Can you work these out from the model? Positions are in its coordinate system, mm. A direction names the side the tool comes from. Coordinates: 2 decimals unless noted, no trailing zeros. Loops run counter-clockwise (first coordinate to the right, second up) from the corner with the lowest first, then second, coordinate; pieces in that order, holes last.
```python
from build123d import *

# Parameters (mm, degrees)
SKETCH1_R                                           = 90
SKETCH1_R_2                                         = 35
BOSS_EXTRUDE1_DEPTH                                 = 20
CUT_EXTRUDE1_DEPTH                                  = 10
CHAMFER1_SIZE                                       = 5
CSK_FOR_1_4_FLAT_HEAD_MACHINE_SCREW_100_D           = 7.14248
CSK_FOR_1_4_FLAT_HEAD_MACHINE_SCREW_100_CSINK_D     = 12.8778
CSK_FOR_1_4_FLAT_HEAD_MACHINE_SCREW_100_CSINK_ANGLE = 100
MIRROR2_COPY_1_D                                    = 7.14248
MIRROR2_COPY_1_CSINK_D                              = 12.8778
MIRROR2_COPY_1_CSINK_ANGLE                          = 100


with BuildPart() as part:
    # Sketch1 → Boss-Extrude1 (new body)
    with BuildSketch(Plane.XY):
        Circle(SKETCH1_R)
        Circle(SKETCH1_R_2, mode=Mode.SUBTRACT)
    extrude(amount=BOSS_EXTRUDE1_DEPTH)

    # Sketch2 → Cut-Extrude1 (cut)
    with BuildSketch(Plane.XY.offset(20)):
        with BuildLine():
            Line((-19.468288874, 43.327078465), (-30.54243357, 66.327225141))
            ThreePointArc((-30.54243357, 66.327225141), (-53.118804443, 50.105225854), (-67.996083401, 26.620925706))
            Line((-67.996083401, 26.620925706), (-43.882710923, 18.181245339))
            ThreePointArc((-43.882710923, 18.181245339), (-34.079547015, 33.088283051), (-19.468288874, 43.327078465))
        make_face()
        with BuildLine():
            Line((43.882710923, 18.181245339), (67.996083401, 26.620925706))
            ThreePointArc((67.996083401, 26.620925706), (53.118804443, 50.105225854), (30.54243357, 66.327225141))
            Line((30.54243357, 66.327225141), (19.468288874, 43.327078465))
            ThreePointArc((19.468288874, 43.327078465), (34.079547015, 33.088283051), (43.882710923, 18.181245339))
        make_face()
        with BuildLine():
            Line((19.468288874, -43.327078465), (30.54243357, -66.327225141))
            ThreePointArc((30.54243357, -66.327225141), (53.118804443, -50.105225854), (67.996083401, -26.620925706))
            Line((67.996083401, -26.620925706), (43.882710923, -18.181245339))
            ThreePointArc((43.882710923, -18.181245339), (34.079547015, -33.088283051), (19.468288874, -43.327078465))
        make_face()
        with BuildLine():
            Line((-43.882710923, -18.181245339), (-67.996083401, -26.620925706))
            ThreePointArc((-67.996083401, -26.620925706), (-53.118804443, -50.105225854), (-30.54243357, -66.327225141))
            Line((-30.54243357, -66.327225141), (-19.468288874, -43.327078465))
            ThreePointArc((-19.468288874, -43.327078465), (-34.079547015, -33.088283051), (-43.882710923, -18.181245339))
        make_face()
    extrude(amount=-CUT_EXTRUDE1_DEPTH, mode=Mode.SUBTRACT)

    # Chamfer1
    chamfer1_edges = [part.edges().sort_by_distance(p)[0] for p in [
        (-90, 0, 20),
    ]]
    chamfer(chamfer1_edges, length=CHAMFER1_SIZE)

    # CSK for 1/4 Flat Head Machine Screw (100)1 (through all)
    with Locations(Plane.XY.offset(10)):
        with Locations((-42.426406871, 42.426406871)):
            csk_for_1_4_flat_head_machine_screw_100 = CounterSinkHole(CSK_FOR_1_4_FLAT_HEAD_MACHINE_SCREW_100_D / 2, CSK_FOR_1_4_FLAT_HEAD_MACHINE_SCREW_100_CSINK_D / 2, counter_sink_angle=CSK_FOR_1_4_FLAT_HEAD_MACHINE_SCREW_100_CSINK_ANGLE)

    # Mirror1: CSK for 1/4 Flat Head Machine Screw (100)1 across plane
    add(csk_for_1_4_flat_head_machine_screw_100.mirror(Plane(origin=(0, 0, 0), x_dir=(0, 0, 1), z_dir=(1, 0, 0))), mode=Mode.SUBTRACT)

    # Mirror2: CSK for 1/4 Flat Head Machine Screw (100)1 across plane
    add(csk_for_1_4_flat_head_machine_screw_100.mirror(Plane.ZX), mode=Mode.SUBTRACT)

    # Mirror2 copy 1 (through all)
    with Locations(Plane(origin=(0, 0, 10), x_dir=(-1, 0, 0), z_dir=(0, 0, 1))):
        with Locations((-42.426406871, 42.426406871)):
            CounterSinkHole(MIRROR2_COPY_1_D / 2, MIRROR2_COPY_1_CSINK_D / 2, counter_sink_angle=MIRROR2_COPY_1_CSINK_ANGLE)


solid = part.part
```
Item 1: Suppose I cut it at A-A, the plane x = 0. Please give me the cut outline in (y, z), plus the area to 4 significant figures.
Results are:
outline: (-90, 0) - (-35, 0) - (-35, 20) - (-85, 20) - (-90, 15) - close; (35, 0) - (90, 0) - (90, 15) - (85, 20) - (35, 20) - close
area: 2,175 mm2
Item 2: I'm going to push flat-ended pins straight in: P1, Ø10, axis at x = -61.5, z = 12, coming from the -Y side; P2, Ø12, axis at y = 40.5, z = 15.5, coming from the -X side; P3, Ø10, axis at x = -1.5, y = 25, coming from the -Z side; P4, Ø3, axis at x = 12, z = 14, coming from the +Y side. Where does each tip first touch, or does it pass through?
Results are:
P1: stops at y = -70.06
P2: stops at x = -83.12
P3: passes through
P4: stops at y = 89.39
Item 3: I need wall thicknesses on line 1 along X through (y, z) = (42, 9); line 2 along X through (y, z) = (-41.5, 10.5); line 3 along Y through (x, z) = (-26.5, 12). Which ranges of each line are inside material? Lowest first, please.
Results are:
line 1: x = -79.6 to -47.66, -37.2 to 37.2, 47.66 to 79.6
line 2: x = -79.86 to -60.08, -23.11 to 23.11, 60.08 to 79.86
line 3: y = -86.01 to -57.93, -39.42 to -22.86, 22.86 to 39.42, 57.93 to 86.01
Item 4: On a 3-axis mill with a long thin cutter (end or side, diameter ignored), from which of +Z, -Z, +X, -X, +Y, -Y can I reach the whole of each face in a straight line? I mean faces 5 (the face through (39, 1, 0)), 6 (the face through (49, -37, 10)). Say none if no direction works.
Results are:
face 5: -Z, +X, -X, +Y, -Y
face 6: +Z
Item 5: Suppose I cut it at C-C, the plane z = 4.25. Please give me the cut outline in (x, y), plus the area to 3 significant figures.
Results are:
outline: circle Ø180 at (0, 0); hole circle Ø7.14 at (-42.43, -42.43); hole circle Ø7.14 at (-42.43, 42.43); hole circle Ø70 at (0, 0); hole circle Ø7.14 at (42.43, -42.43); hole circle Ø7.14 at (42.43, 42.43)
area: 21,400 mm2
Item 6: We'd pull the mould along Y, two halves only. Please class faces 1 (the face through (-49, 43, 10)), 2 (the face through (52.85, -50.39, 15.07)), 3 (the face through (41.53, -79.845, 7.395)), 4 (the face through (-1, -37, 20)): +Y half, -Y half, draft (parallel to the pull), parting line (faces both ways), or undercut.
Results are:
face 1: undercut
face 2: undercut
face 3: parting line
face 4: draft
